from build123d import *

# Parameters (mm, degrees)
SKETCH_1_W          = 20
SKETCH_1_H          = 10
EXTRUDE_1_DEPTH     = 9.5
SKETCH_2_W          = 16.2
SKETCH_2_H          = 29.89512134
CUT_EXTRUDE_1_DEPTH = 2.2
CUT_EXTRUDE_2_DEPTH = 23.699118926


with BuildPart() as part:
    # 草图1 → 凸台-拉伸1 (new body)
    with BuildSketch(Plane.XY):
        Rectangle(SKETCH_1_W, SKETCH_1_H)
    extrude(amount=EXTRUDE_1_DEPTH)

    # 草图2 → 切除-拉伸1 (cut)
    with BuildSketch(Plane.XY.offset(9.5)):
        Rectangle(SKETCH_2_W, SKETCH_2_H)
    extrude(amount=-CUT_EXTRUDE_1_DEPTH, mode=Mode.SUBTRACT)

    # 草图3 → 切除-拉伸2 (cut, through all)
    with BuildSketch(Plane.ZY.offset(10)):
        Polygon((0, 5), (3.5, 5), (0, 1.5), align=None)
    cut_extrude_2 = extrude(amount=-CUT_EXTRUDE_2_DEPTH, mode=Mode.SUBTRACT)

    # 镜向1: 切除-拉伸2 across plane
    add(cut_extrude_2.mirror(Plane.ZX), mode=Mode.SUBTRACT)


solid = part.part
Can you work these out from the model? Positions are in its coordinate system, mm. A direction names the side the tool comes from. Round coordinates to 2 decimals unless told otherwise and drop trailing zeros. Order: outer loops, then holes, each group sorted by start corner. A loop starts at its lowest first (then second) coordinate and runs counter-clockwise, first axis right, second up. Notation, with made-up numbers: (83, 46) - (112, 46) arc R23 ccw to (112, 57) - close; hole circle Ø4 at (-30, 66). An arc over 180 degrees is marked (long way). Answer in a Markdown table with one row per item.
(1) Suppose I cut it at C-C, the plane x = 3. Please give me the cut outline in (y, z).
From the geometry:
| item | result |
|---|---|
| outline | (-5, 3.5) - (-1.5, 0) - (1.5, 0) - (5, 3.5) - (5, 7.3) - (-5, 7.3) - close |
(2) If we mould it in two halves opening along X, with no side actions, what happens to faces 1 (the face through (10, 0, 6)), 2 (the face through (8.1, 0, 8)), 3 (the face through (-9, 0, 9.5))? For each: released by +X, released by -X, zero draft, split by the parting line, or undercut.
From the geometry:
| item | result |
|---|---|
| face 1 | released by +X |
| face 2 | undercut |
| face 3 | zero draft |
(3) Suppose I cut it at D-D, the plane y = 2.75. Please give me the cut outline in (x, z), plus the area to 3 significant figures.
From the geometry:
| item | result |
|---|---|
| outline | (-10, 1.25) - (10, 1.25) - (10, 9.5) - (8.1, 9.5) - (8.1, 7.3) - (-8.1, 7.3) - (-8.1, 9.5) - (-10, 9.5) - close |
| area | 129 mm2 |
(4) Suppose I cut it at A-A, the plane z = 7.5. Please give me the cut outline in (x, y).
From the geometry:
| item | result |
|---|---|
| outline | (-10, -5) - (-8.1, -5) - (-8.1, 5) - (-10, 5) - close; (8.1, -5) - (10, -5) - (10, 5) - (8.1, 5) - close |
(5) Please list where these lines run through material, in increasing order: L1, parallel to X at y = 2.75, z = 7.5; L2, parallel to Z at x = 3, y = -1; L3, parallel to Z at x = -2.5, y = 3. Write a range as from..to.
From the geometry:
| item | result |
|---|---|
| L1 | x = -10..-8.1, 8.1..10 |
| L2 | z = 0..7.3 |
| L3 | z = 1.5..7.3 |
(6) Suppose I cut it at B-B, the plane y = -1.75. Please give me the cut outline in (x, z).
From the geometry:
| item | result |
|---|---|
| outline | (-10, 0.25) - (10, 0.25) - (10, 9.5) - (8.1, 9.5) - (8.1, 7.3) - (-8.1, 7.3) - (-8.1, 9.5) - (-10, 9.5) - close |
(7) Which directions (+Z, -Z, +X, -X, +Y, -Y) give clear straight access to the entire face, cutting with the end or side of a thin tool? Please do faces 4 (the face through (-8.1, 0, 8)), 5 (the face through (9, 0, 9.5)).
From the geometry:
| item | result |
|---|---|
| face 4 | +Z, +Y, -Y |
| face 5 | +Z, +X, -X, +Y, -Y |
(8) For P1, Ø2, axis at x = -6.5, y = 2, coming from the +Z side, with a flat end and sliding along its axis, tell me the tip position at first contact or that it passes through.
From the geometry:
| item | result |
|---|---|
| P1 | stops at z = 7.3 |
